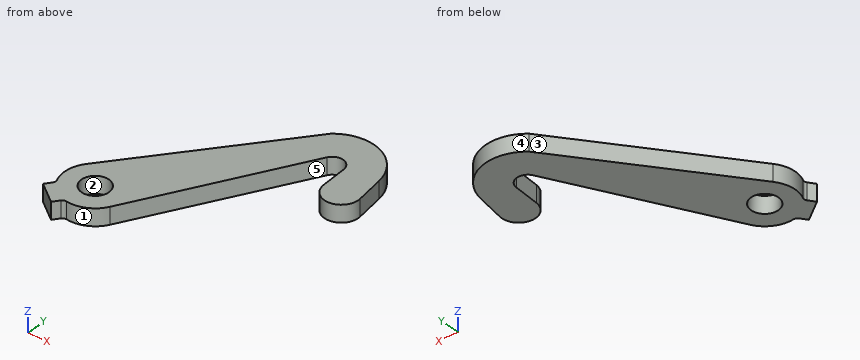
```python
from build123d import *

# Parameters (mm, degrees)
SKETCH1_R           = 6.5
BOSS_EXTRUDE1_DEPTH = 4
FILLET1_R           = 2


with BuildPart() as part:
    # Sketch1 → Boss-Extrude1 (new, symmetric)
    with BuildSketch(Plane.XY):
        with BuildLine():
            Line((47.613190214, 66.596790509), (6.61525122, -8.614210923))
            ThreePointArc((6.61525122, -8.614210923), (-0.051073307, -14.850717485), (-9.121738509, -15.878788295))
            Line((-9.121738509, -15.878788295), (-12.077727744, -19.911421137))
            Line((-12.077727744, -19.911421137), (-21.756046565, -12.817046972))
            Line((-21.756046565, -12.817046972), (-18.80005733, -8.784414129))
            ThreePointArc((-18.80005733, -8.784414129), (-20.623291354, -0.545508517), (-17.559429464, 7.316838354))
            Line((-17.559429464, 7.316838354), (39.076322986, 79.353992026))
            ThreePointArc((39.076322986, 79.353992026), (59.174366459, 82.937056923), (72.02582234, 67.074844364))
            Line((72.02582234, 67.074844364), (74.007984491, 53.75944084))
            ThreePointArc((74.007984491, 53.75944084), (66.847485005, 44.555404253), (57.99070376, 52.141211286))
            Line((57.99070376, 52.141211286), (57.333258746, 64.39522394))
            ThreePointArc((57.333258746, 64.39522394), (53.305241341, 69.169419157), (47.613190214, 66.596790509))
        make_face()
        with Locations((-6.139534384, -1.661505705)):
            Circle(SKETCH1_R, mode=Mode.SUBTRACT)
    extrude(amount=BOSS_EXTRUDE1_DEPTH, both=True)

    # Fillet1
    fillet1_edges = [part.edges().sort_by_distance(p)[0] for p in [
        (-18.80005733, -8.784414129, 0),
        (-9.121738509, -15.878788295, 0),
    ]]
    fillet(fillet1_edges, radius=FILLET1_R)


solid = part.part
```
Work out the finished part from the listing and answer in its coordinate system (mm). Face numbers are marked on the shaded views. A direction names the side the tool comes from. Round coordinates to 2 decimals unless told otherwise and drop trailing zeros. Order: outer loops, then holes, each group sorted by start corner. A loop starts at its lowest first (then second) coordinate and runs counter-clockwise, first axis right, second up.
Q1. A cutting plane is placed at A-A, the plane y = -5.5. Determine the outline of the cut face in (x, z).
Solution:
outline: (-20.15, -4) - (-11.39, -4) - (-11.39, 4) - (-20.15, 4) - close; (-0.89, -4) - (8.31, -4) - (8.31, 4) - (-0.89, 4) - close
Q2. A cutting plane is placed at D-D, the plane x = 36. Determine the outline of the cut face in (y, z), then the cut area to 3 significant figures.
Solution:
outline: (45.29, -4) - (75.44, -4) - (75.44, 4) - (45.29, 4) - close
area: 241 mm2
Q3. A tool of negligible diameter and unlimited length cuts with its end or side. For the marked faces 4 and 5, from which of +Z, -Z, +X, -X, +Y, -Y can it reach the whole face along a straight path? Write none if from no direction.
Solution:
face 4: +Z, -Z, +Y
face 5: +Z, -Z, -Y
Q4. Find the intervals of material crossed by line 1 along X through (y, z) = (-5.5, -2.25); line 2 along X through (y, z) = (50.5, 2.25); line 3 along Y through (x, z) = (68, 1), in increasing order.
Solution:
line 1: x = -20.15 to -11.39, -0.89 to 8.31
line 2: x = 16.39 to 38.84, 58.25 to 73.82
line 3: y = 44.76 to 76.47
Q5. The mould has two halves that part along Y. Classify the marked faces 1, 2 and 3: pulls with the +Y half, pulls with the -Y half, needs draft (parallel to the pull), parting line crosses it, or undercut.
Solution:
face 1: pulls with the -Y half
face 2: undercut
face 3: pulls with the +Y half
Q6. A cutting plane is placed at C-C, the plane y = 48.5. Determine the outline of the cut face in (x, z).
Solution:
outline: (14.82, -4) - (37.75, -4) - (37.75, 4) - (14.82, 4) - close; (59.08, -4) - (72.99, -4) - (72.99, 4) - (59.08, 4) - close
Q7. A cutting plane is placed at B-B, the plane z = -2.5. Determine the outline of the cut face in (x, y), then the cut area to 3 significant figures.
Solution:
outline: (-21.76, -12.82) - (-12.08, -19.91) - (-9.85, -16.87) arc R2 cw to (-7.98, -16.07) arc R14.53 ccw to (6.62, -8.61) - (47.61, 66.6) arc R5.18 cw to (57.33, 64.4) - (57.99, 52.14) arc R8.06 ccw (long way) to (74.01, 53.76) - (72.03, 67.07) arc R20.08 ccw to (39.08, 79.35) - (-17.56, 7.32) arc R14.53 ccw to (-19.33, -7.76) arc R2 cw to (-19.53, -9.78) - close; hole circle Ø13 at (-6.14, -1.66)
area: 2,910 mm2
Q8. Given pin 1 Ø2 at (y, z) = (17, 2) entering from -X; pin 2 Ø3 at (y, z) = (11.5, 2.5) entering from +X; pin 3 Ø2 at (x, z) = (63, 3) entering from +Y, each flat-ended and moving along its own axis, determine where each tip first touches the part or whether it passes through.
Solution:
pin 1: stops at x = -10.73
pin 2: stops at x = 18.4
pin 3: stops at y = 81.63
